Input: part model. Units: mm. Frame: model coordinates. A direction names the side the tool comes from. Give positions to 0.01 mm unless a question says otherwise; leave off trailing zeros. Loops run counter-clockwise (first coordinate to the right, second up) from the corner with the lowest first, then second, coordinate; pieces in that order, holes last. Notation, with made-up numbers: (34, 53.25) - (51, 53.25) arc R21 ccw to (51, 70.25) - close; hole circle Ø8 at (43, -8). An arc over 180 degrees is marked (long way). One line per item, written item: value.
from build123d import *

# Parameters (mm, degrees)
SKETCH_1_W          = 8
SKETCH_1_H          = 8
SKETCH_1_W_2        = 6
SKETCH_1_H_2        = 6
EXTRUDE_1_DEPTH     = 152
SKETCH_2_R          = 1.55
CUT_EXTRUDE_1_DEPTH = 153.262930485
SKETCH_3_R          = 1.55
CUT_EXTRUDE_2_DEPTH = 153.262930485


with BuildPart() as part:
    # 草图1 → 凸台-拉伸1 (new body)
    with BuildSketch(Plane(origin=(0, 0, 0), x_dir=(1, 0, 0), z_dir=(0, 1, 0))):
        Rectangle(SKETCH_1_W, SKETCH_1_H)
        Rectangle(SKETCH_1_W_2, SKETCH_1_H_2, mode=Mode.SUBTRACT)
    extrude(amount=EXTRUDE_1_DEPTH)

    # 草图2 → 切除-拉伸1 (cut, through all)
    with BuildSketch(Plane.XY.offset(4)):
        with Locations((0, 147)):
            Circle(SKETCH_2_R)
        with Locations((0, 4)):
            Circle(SKETCH_2_R)
        with Locations((0, 12)):
            Circle(SKETCH_2_R)
    extrude(amount=-CUT_EXTRUDE_1_DEPTH, mode=Mode.SUBTRACT)

    # 草图3 → 切除-拉伸2 (cut, through all)
    with BuildSketch(Plane(origin=(4, 0, 0), x_dir=(0, 0, -1), z_dir=(1, 0, 0))):
        with Locations((0, 135)):
            Circle(SKETCH_3_R)
        with Locations((0, 20)):
            Circle(SKETCH_3_R)
        with Locations((0, 110)):
            Circle(SKETCH_3_R)
        with Locations((0, 80)):
            Circle(SKETCH_3_R)
    extrude(amount=-CUT_EXTRUDE_2_DEPTH, mode=Mode.SUBTRACT)


solid = part.part
Item 1: Section B-B, the plane x = 0. Count the separate pieces of the cut face and the enclosed holes in it, and give its area (3 significant figures).
Verdict:
separate pieces: 8
enclosed holes: 0
area: 285 mm^2
Item 2: Section C-C, the plane y = 24.5. Output: boundary loops of the cut face in (x, z).
Verdict:
outline: (-4, -4) - (4, -4) - (4, 4) - (-4, 4) - close; hole (-3, -3) - (3, -3) - (3, 3) - (-3, 3) - close
Item 3: Draft query along Z for faces 3 (the face through (-3.493, 108.487, 0.336)), 4 (the face through (-0.336, 145.487, 3.507)), 5 (the face through (0, 75, 4)), 6 (the face through (3.507, 133.487, 0.336)). Return one class per face: pulls with the +Z half, pulls with the -Z half, needs draft (parallel to the pull), parting line crosses it, or undercut.
Verdict:
face 3: undercut
face 4: needs draft
face 5: pulls with the +Z half
face 6: undercut
Item 4: Access query for faces 1 (the face through (3, 75, 0)), 2 (the face through (-4, 75, 0)). Directions: +Z, -Z, +X, -X, +Y, -Y. A direction counts if a zero-diameter tool reaches every point of the face in a straight line with its end or side. Return the directions, or none.
Verdict:
face 1: +Y, -Y
face 2: +Z, -Z, -X, +Y, -Y
Item 5: Section A-A, the plane y = 80. Output: boundary loops of the cut face in (x, z), and give its area (3 significant figures).
Verdict:
outline: (-4, -4) - (4, -4) - (4, -1.55) - (3, -1.55) - (3, -3) - (-3, -3) - (-3, -1.55) - (-4, -1.55) - close; (-4, 1.55) - (-3, 1.55) - (-3, 3) - (3, 3) - (3, 1.55) - (4, 1.55) - (4, 4) - (-4, 4) - close
area: 21.8 mm^2
Item 6: Pin query (flat end, axial travel): P1, Ø3.5, axis at y = 20, z = 0, coming from the +X side. Return the tip coordinate at first contact, or that it passes through.
Verdict:
P1: stops at x = 4
Item 7: Material intervals for L1, parallel to Y at x = -3.8, z = 0; L2, parallel to Y at x = 0, z = 3.7; L3, parallel to Z at x = 1, y = 31, sorted ascending.
Verdict:
L1: y = 0 to 18.45, 21.55 to 78.45, 81.55 to 108.45, 111.55 to 133.45, 136.55 to 152
L2: y = 0 to 2.45, 5.55 to 10.45, 13.55 to 145.45, 148.55 to 152
L3: z = -4 to -3, 3 to 4
